from build123d import *

# Parameters (mm, degrees)
BASE_BLOCK_PROFILE_W      = 50
BASE_BLOCK_PROFILE_H      = 40
BASE_BLOCK_50X40X40_DEPTH = 20
STEP_CUT_1_DEPTH          = 10
STEP_CUT_2_DEPTH          = 10
STEP_CUT_3_DEPTH          = 10


with BuildPart() as part:
    # Base Block Profile → Base Block 50x40x40 (new, symmetric)
    with BuildSketch(Plane(origin=(0, 0, 0), x_dir=(1, 0, 0), z_dir=(0, 1, 0))):
        Rectangle(BASE_BLOCK_PROFILE_W, BASE_BLOCK_PROFILE_H)
    extrude(amount=BASE_BLOCK_50X40X40_DEPTH, both=True)

    # Step Cut 1 Profile → Step Cut 1 (cut)
    with BuildSketch(Plane(origin=(0, 20, 0), x_dir=(1, 0, 0), z_dir=(0, 1, 0))):
        Polygon((25, 20), (15, 0), (5, 0), (-5, -20), (25, -20), align=None)
    extrude(amount=-STEP_CUT_1_DEPTH, mode=Mode.SUBTRACT)

    # Step Cut 2 Profile → Step Cut 2 (cut)
    with BuildSketch(Plane(origin=(0, 10, 0), x_dir=(1, 0, 0), z_dir=(0, 1, 0))):
        Polygon((25, 0), (15, 0), (5, -20), (25, -20), align=None)
    extrude(amount=-STEP_CUT_2_DEPTH, mode=Mode.SUBTRACT)

    # Step Cut 3 Profile → Step Cut 3 (cut)
    with BuildSketch(Plane(origin=(0, 0, 0), x_dir=(1, 0, 0), z_dir=(0, 1, 0))):
        Polygon((25, -20), (25, 0), (15, -20), align=None)
    extrude(amount=-STEP_CUT_3_DEPTH, mode=Mode.SUBTRACT)


solid = part.part
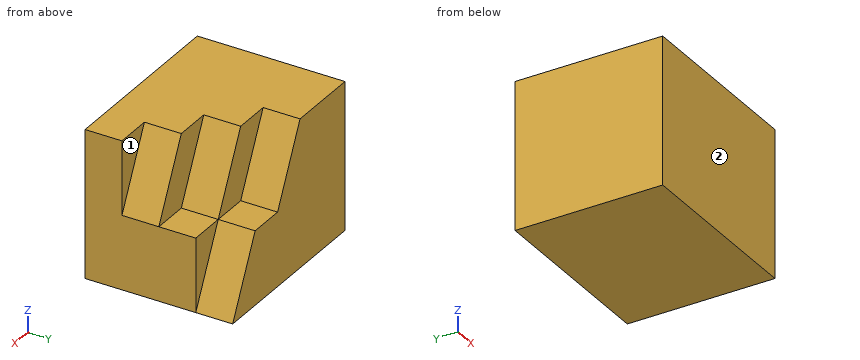
Design review of the part built by this model. Coordinates are the model's own, in mm. Face numbers are marked on the shaded views. A direction names the side the tool comes from. Coordinates: 2 decimals unless noted, no trailing zeros. Order: outer loops, then holes, each group sorted by start corner. A loop starts at its lowest first (then second) coordinate and runs counter-clockwise, first axis right, second up.
Item 1: For line 1 (Y direction, x = 6, z = 10); line 2 (Y direction, x = 11.5, z = 11), list the stretches that pass through material, from the lowest coordinate up.
Item 2: Take a section at B-B, the plane x = 13.5. Write out the cut boundary in (y, z).
Item 3: For pin 1 Ø12 at (y, z) = (-2, 8.5) entering from +X; pin 2 Ø5 at (x, z) = (21.5, 8) entering from +Y; pin 3 Ø3 at (x, y) = (10.5, 16.5) entering from +Z, all flat-tipped, find the tip position at first contact; note any pin that passes through.
Item 4: Take a section at A-A, the plane z = 2. Write out the cut boundary in (x, y).
Item 5: Take a section at D-D, the plane z = 12.5. Write out the cut boundary in (x, y), then the cut area to 3 significant figures.
Item 6: Take a section at C-C, the plane y = 6.5. Write out the cut boundary in (x, z), then the cut area to 3 significant figures.
Item 7: For the marked faces 1 and 2, list the 3-axis set-ups (+Z, -Z, +X, -X, +Y, -Y) from which the entire face can be reached by the end or side of a thin tool; tool diameter is ignored.
The answers:
1. line 1: y = -20 to 10
1. line 2: y = -20 to 0
2. outline: (-20, -20) - (20, -20) - (20, 0) - (10, 0) - (10, 3) - (0, 3) - (0, 20) - (-20, 20) - close
3. pin 1: stops at x = 23.75
3. pin 2: stops at y = 0
3. pin 3: stops at z = 0
4. outline: (-25, -20) - (25, -20) - (25, -10) - (24, -10) - (24, 0) - (14, 0) - (14, 10) - (4, 10) - (4, 20) - (-25, 20) - close
5. outline: (-25, -20) - (25, -20) - (25, -10) - (18.75, -10) - (18.75, 0) - (8.75, 0) - (8.75, 10) - (-1.25, 10) - (-1.25, 20) - (-25, 20) - close
5. area: 1,510 mm2
6. outline: (-25, -20) - (25, -20) - (25, 0) - (15, 0) - (5, 20) - (-25, 20) - close
6. area: 1,700 mm2
7. face 1: +Z, +X, +Y
7. face 2: +Z, -Z, +X, -X, -Y
